The drawing under review shows one solid part. Ordinate dimensions are in mm from its lowest x, y, z. Give positions to 0.01 mm unless a question says otherwise; leave off trailing zeros. Order: outer loops, then holes, each group sorted by start corner. A loop starts at its lowest first (then second) coordinate and runs counter-clockwise, first axis right, second up. Notation, with made-up numbers: (-31, 70.25) -> (28, 70.25) arc R24 ccw to (28, 92.25) -> close; hole circle Ø5 at (-31, 87). An arc over 180 degrees is marked (long way). Use CSV: the item, a comma, the result in double quotes. Start each with the question number.
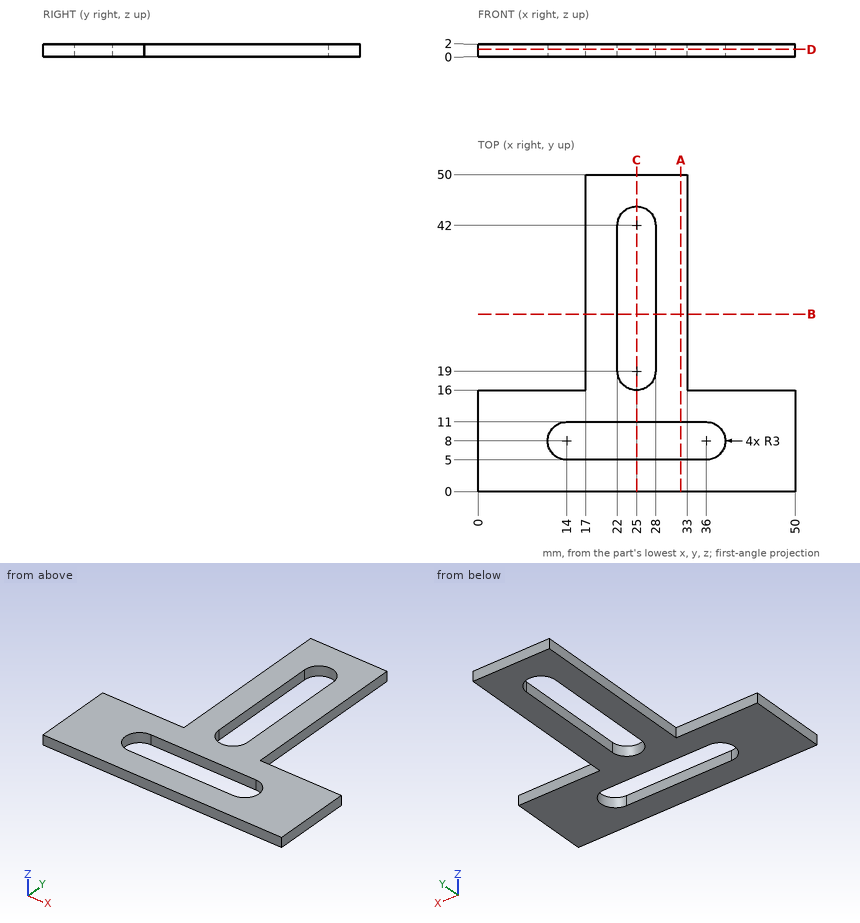
1. Clearance check with flat-ended pins moving along their axes: P1, Ø1, axis at y = 26.5, z = 1, coming from the -X side; P2, Ø1, axis at x = 6.5, z = 1, coming from the +Y side; P3, Ø1, axis at y = 28, z = 0.5, coming from the +X side. State where each tip first meets the part, or that it passes through.
2. To check wall thickness, follow L1, parallel to X at y = 36, z = 1.5; L2, parallel to Y at x = 17.5, z = 1.55; L3, parallel to Y at x = 15, z = 1.8. State the ranges of each line that lie inside material, in increasing order. Write a range as [from, to].
3. Consider section D-D (z = 1.15). State the section outline as (x, y) points.
4. Consider section B-B (y = 28). State the section outline as (x, z) points.
5. Consider section A-A (x = 32). State the section outline as (y, z) points.
6. Consider section C-C (x = 25). State the section outline as (y, z) points, plus the area to 3 significant figures.
Answer list:
1,P1,"x = 17"
1,P2,"y = 16"
1,P3,"x = 33"
2,L1,"[17, 22], [28, 33]"
2,L2,"[0, 5], [11, 50]"
2,L3,"[0, 5], [11, 16]"
3,outline,"(0, 0) -> (50, 0) -> (50, 16) -> (33, 16) -> (33, 50) -> (17, 50) -> (17, 16) -> (0, 16) -> close; hole (14, 5) -> (36, 5) arc R3 ccw to (36, 11) -> (14, 11) arc R3 ccw to start; hole (22, 19) arc R3 ccw to (28, 19) -> (28, 42) arc R3 ccw to (22, 42) -> close"
4,outline,"(17, 0) -> (22, 0) -> (22, 2) -> (17, 2) -> close; (28, 0) -> (33, 0) -> (33, 2) -> (28, 2) -> close"
5,outline,"(0, 0) -> (5, 0) -> (5, 2) -> (0, 2) -> close; (11, 0) -> (50, 0) -> (50, 2) -> (11, 2) -> close"
6,outline,"(0, 0) -> (5, 0) -> (5, 2) -> (0, 2) -> close; (11, 0) -> (16, 0) -> (16, 2) -> (11, 2) -> close; (45, 0) -> (50, 0) -> (50, 2) -> (45, 2) -> close"
6,area,"30.0 mm2"
